Geometry check sheet. Reference: the model listing, model coordinates, mm. Coordinates: 2 decimals unless noted, no trailing zeros. Loops run counter-clockwise (first coordinate to the right, second up) from the corner with the lowest first, then second, coordinate; pieces in that order, holes last. Notation, with made-up numbers: M 72.25,-14.5 L 97.25,-14.5 A10 ccw 97.25,-1.5 Z; hole C 85,89.25 d11. An arc over 180 degrees is marked long. Use CSV: the item, a comma, the result in double quotes.
```python
from build123d import *

# Parameters (mm, degrees)
SKETCH1_R                 = 2.65
F_30_X_60G_X_R1_5_1_DEPTH = 600


with BuildPart() as part:
    # Sketch1 → 工业铝型材 30 X 60G X R1.5(1) (new body)
    with BuildSketch(Plane.YZ.offset(-300)):
        with BuildLine():
            Line((-3.25, 30), (-3.25, 29))
            Line((-3.25, 29), (-4.25, 29))
            Line((-4.25, 29), (-4.25, 21.277812156))
            ThreePointArc((-4.25, 21.277812156), (0, 20.5), (4.25, 21.277812156))
            Line((4.25, 21.277812156), (4.25, 29))
            Line((4.25, 29), (3.25, 29))
            Line((3.25, 29), (3.25, 30))
            Line((3.25, 30), (13.5, 30))
            ThreePointArc((13.5, 30), (14.560660172, 29.560660172), (15, 28.5))
            Line((15, 28.5), (15, 18.25))
            Line((15, 18.25), (14, 18.25))
            Line((14, 18.25), (14, 19.25))
            Line((14, 19.25), (6.277812156, 19.25))
            ThreePointArc((6.277812156, 19.25), (5.5, 15), (6.277812156, 10.75))
            Line((6.277812156, 10.75), (14, 10.75))
            Line((14, 10.75), (14, 11.75))
            Line((14, 11.75), (15, 11.75))
            Line((15, 11.75), (15, -11.75))
            Line((15, -11.75), (14, -11.75))
            Line((14, -11.75), (14, -10.75))
            Line((14, -10.75), (6.277812156, -10.75))
            ThreePointArc((6.277812156, -10.75), (5.5, -15), (6.277812156, -19.25))
            Line((6.277812156, -19.25), (14, -19.25))
            Line((14, -19.25), (14, -18.25))
            Line((14, -18.25), (15, -18.25))
            Line((15, -18.25), (15, -28.5))
            ThreePointArc((15, -28.5), (14.560660172, -29.560660172), (13.5, -30))
            Line((13.5, -30), (3.25, -30))
            Line((3.25, -30), (3.25, -29))
            Line((3.25, -29), (4.25, -29))
            Line((4.25, -29), (4.25, -21.277812156))
            ThreePointArc((4.25, -21.277812156), (0, -20.5), (-4.25, -21.277812156))
            Line((-4.25, -21.277812156), (-4.25, -29))
            Line((-4.25, -29), (-3.25, -29))
            Line((-3.25, -29), (-3.25, -30))
            Line((-3.25, -30), (-13.5, -30))
            ThreePointArc((-13.5, -30), (-14.560660172, -29.560660172), (-15, -28.5))
            Line((-15, -28.5), (-15, -18.25))
            Line((-15, -18.25), (-14, -18.25))
            Line((-14, -18.25), (-14, -19.25))
            Line((-14, -19.25), (-6.277812156, -19.25))
            ThreePointArc((-6.277812156, -19.25), (-5.5, -15), (-6.277812156, -10.75))
            Line((-6.277812156, -10.75), (-14, -10.75))
            Line((-14, -10.75), (-14, -11.75))
            Line((-14, -11.75), (-15, -11.75))
            Line((-15, -11.75), (-15, 11.75))
            Line((-15, 11.75), (-14, 11.75))
            Line((-14, 11.75), (-14, 10.75))
            Line((-14, 10.75), (-6.277812156, 10.75))
            ThreePointArc((-6.277812156, 10.75), (-5.5, 15), (-6.277812156, 19.25))
            Line((-6.277812156, 19.25), (-14, 19.25))
            Line((-14, 19.25), (-14, 18.25))
            Line((-14, 18.25), (-15, 18.25))
            Line((-15, 18.25), (-15, 28.5))
            ThreePointArc((-15, 28.5), (-14.560660172, 29.560660172), (-13.5, 30))
            Line((-13.5, 30), (-3.25, 30))
        make_face()
        with Locations((-11, 26)):
            Circle(SKETCH1_R, mode=Mode.SUBTRACT)
        with Locations((11, 26)):
            Circle(SKETCH1_R, mode=Mode.SUBTRACT)
        with Locations((11, -26)):
            Circle(SKETCH1_R, mode=Mode.SUBTRACT)
        with Locations((-11, -26)):
            Circle(SKETCH1_R, mode=Mode.SUBTRACT)
        with BuildLine():
            Line((-12.5, 7.5), (-4, 7.5))
            Line((-4, 7.5), (-1.665625283, 13.135679101))
            ThreePointArc((-1.665625283, 13.135679101), (0, 17.5), (1.665625283, 13.135679101))
            Line((1.665625283, 13.135679101), (4, 7.5))
            Line((4, 7.5), (12.5, 7.5))
            Line((12.5, 7.5), (12.5, -7.5))
            Line((12.5, -7.5), (4, -7.5))
            Line((4, -7.5), (1.665625283, -13.135679101))
            ThreePointArc((1.665625283, -13.135679101), (0, -17.5), (-1.665625283, -13.135679101))
            Line((-1.665625283, -13.135679101), (-4, -7.5))
            Line((-4, -7.5), (-12.5, -7.5))
            Line((-12.5, -7.5), (-12.5, 7.5))
        make_face(mode=Mode.SUBTRACT)
    extrude(amount=F_30_X_60G_X_R1_5_1_DEPTH)


solid = part.part
```
1. Thickness scan on line 1 (Z direction, x = -157, y = 11); line 2 (Z direction, x = -76, y = -8); line 3 (Y direction, x = -86.5, z = -15). Record the ranges inside material, lowest first. Write a range as [from, to].
The answers:
line 1,"[-30, -28.65], [-23.35, -19.25], [-10.75, -7.5], [7.5, 10.75], [19.25, 23.35], [28.65, 30]"
line 2,"[-30, -19.25], [-10.75, -7.5], [7.5, 10.75], [19.25, 30]"
line 3,"[-5.5, -2.5], [2.5, 5.5]"
2. Section check A-A, the plane z = -2. Record the cut outline in (x, y), plus the area to 3 significant figures.
The answers:
outline,"M -300,-15 L 300,-15 L 300,-12.5 L -300,-12.5 Z; M -300,12.5 L 300,12.5 L 300,15 L -300,15 Z"
area,"3,000 mm^2"
3. Gauge pin test, flat ends, axial feed: P1, Ø1.5, axis at x = -27, y = 1.5, coming from the +Z side; P2, Ø1.1, axis at x = 35, y = -14.5, coming from the -Z side; P3, Ø3, axis at x = -137, y = 1, coming from the -Z side. Record the tip position at first contact, or that the pin passes through.
The answers:
P1,"z = 20.71"
P2,"z = -29.93"
P3,"z = -20.76"
4. Release check for a two-part mould opening along Z. For faces 1 (the flat face through (-4, -12.5, 0)), 2 (the flat face through (-4, 12.5, 0)), 3 (the flat face through (-4, 8, 30)), 4 (the flat face through (-4, -15, 0)) record: +Z half, -Z half, draft (parallel to the pull), parting line (faces both ways), or undercut.
The answers:
face 1,"undercut"
face 2,"undercut"
face 3,"+Z half"
face 4,"draft"
5. Section check B-B, the plane x = -68.5. Count the separate pieces of the cut face and the enclosed holes in it, plus the area to 3 significant figures.
The answers:
separate pieces,"1"
enclosed holes,"5"
area,"775 mm^2"
